```python
from build123d import *

# Parameters (mm, degrees)
EXTRUDE_1_DEPTH     = 130
SKETCH_2_R          = 3
CUT_EXTRUDE_1_DEPTH = 20
SKETCH_9_W          = 50
SKETCH_9_H          = 55
CUT_EXTRUDE_2_DEPTH = 150
SKETCH_10_W         = 100
SKETCH_10_H         = 45
CUT_EXTRUDE_3_DEPTH = 200


with BuildPart() as part:
    # 草图1 → 凸台-拉伸1 (new body)
    with BuildSketch(Plane.XY):
        with BuildLine():
            Line((-450.427662897, 234.022122697), (-950.427662897, 234.022122697))
            Line((-950.427662897, 234.022122697), (-950.427662897, 299.022122697))
            Line((-950.427662897, 299.022122697), (-450.427662897, 299.022122697))
            ThreePointArc((-450.427662897, 299.022122697), (-217.927662897, 66.522122697), (-450.427662897, -165.977877303))
            Line((-450.427662897, -165.977877303), (-700.427662897, -165.977877303))
            Line((-700.427662897, -165.977877303), (-700.427662897, -100.977877303))
            Line((-700.427662897, -100.977877303), (-450.427662897, -100.977877303))
            ThreePointArc((-450.427662897, -100.977877303), (-282.927662897, 66.522122697), (-450.427662897, 234.022122697))
        make_face()
    extrude(amount=EXTRUDE_1_DEPTH)

    # 草图2 → 切除-拉伸1 (cut)
    with BuildSketch(Plane.ZY.offset(950.427662897)):
        with Locations((6, 279.022122697)):
            Circle(SKETCH_2_R)
        with Locations((6, 254.022122697)):
            Circle(SKETCH_2_R)
        with Locations((124, 279.022122697)):
            Circle(SKETCH_2_R)
        with Locations((124, 254.022122697)):
            Circle(SKETCH_2_R)
    extrude(amount=-CUT_EXTRUDE_1_DEPTH, mode=Mode.SUBTRACT)

    # 草图9 → 切除-拉伸2 (cut)
    with BuildSketch(Plane.XY.offset(130)):
        with Locations((-915.427662897, 266.522122697)):
            Rectangle(SKETCH_9_W, SKETCH_9_H)
    extrude(amount=-CUT_EXTRUDE_2_DEPTH, mode=Mode.SUBTRACT)

    # 草图10 → 切除-拉伸3 (cut)
    with BuildSketch(Plane.ZY.offset(950.427662897)):
        with Locations((65, 266.522122697)):
            Rectangle(SKETCH_10_W, SKETCH_10_H)
    extrude(amount=-CUT_EXTRUDE_3_DEPTH, mode=Mode.SUBTRACT)


solid = part.part
```
Geometry: final body of the model. Coordinates: model frame, mm. A direction names the side the tool comes from. Round coordinates to 2 decimals unless told otherwise and drop trailing zeros. Write each loop counter-clockwise with the first axis right and the second up, starting at its lowest first coordinate (ties: lowest second). Pieces come first, ordered by that corner, then holes. Notation, with made-up numbers: (75, -0.75) -> (118, -0.75) arc R26 cw to (118, 15.25) -> close; hole circle Ø3 at (66.5, 50). An arc over 180 degrees is marked (long way). Return JSON: item names as keys, results as strings.
Q1. Section C-C on x = -377.5. Return the cut outline in (y, z), and give its area (3 significant figures).
From the geometry:
{"outline": "(-154.24, 0) -> (-84.27, 0) -> (-84.27, 130) -> (-154.24, 130) -> close; (217.31, 0) -> (287.29, 0) -> (287.29, 130) -> (217.31, 130) -> close", "area": "18,200 mm2"}
Q2. Set-up query: faces 5 (the flat face through (-916, 294.022, 66)), 6 (the flat face through (-821, 244.022, 64)), 7 (the flat face through (-577, -100.978, 64)). Return all of +Z, -Z, +X, -X, +Y, -Y with unobstructed straight access to the full face (end or side cutting, diameter ignored); none if empty.
From the geometry:
{"face 5": "+Z, -Z", "face 6": "-X", "face 7": "+Z, -Z, -X"}
Q3. First-contact query: pin 1 Ø8 at (y, z) = (279.02, 6) entering from +X; pin 2 Ø3.5 at (y, z) = (279.02, 124) entering from +X; pin 3 Ø9.5 at (y, z) = (254.02, 124) entering from +X. Flat tips, straight axial feed; report the tip coordinate or a pass-through.
From the geometry:
{"pin 1": "x = -347.54", "pin 2": "x = -352.24", "pin 3": "x = -306.69"}
Q4. Mould query, pull axis Z, two halves, no side actions, for faces 1 (the flat face through (-821, 266, 115)), 2 (the flat face through (-750.428, 267, 64)), 3 (the flat face through (-528, 240, 0)), 4 (the flat face through (-574, -165.978, 64)). Classes: +Z half, -Z half, draft (parallel to the pull), parting line (faces both ways), or undercut.
From the geometry:
{"face 1": "undercut", "face 2": "undercut", "face 3": "-Z half", "face 4": "draft"}
Q5. Ray query, line 1 (Y direction, x = -942.25, z = 6); line 2 (Y direction, x = -558.5, z = 112); line 3 (Y direction, x = -914.5, z = 10). Return the intervals inside material, ascending.
From the geometry:
{"line 1": "234.02 to 251.02, 257.02 to 276.02, 282.02 to 299.02", "line 2": "-165.98 to -100.98, 234.02 to 299.02", "line 3": "234.02 to 239.02, 294.02 to 299.02"}
Q6. Section A-A on x = -552. Return the cut outline in (y, z), and give its area (3 significant figures).
From the geometry:
{"outline": "(-165.98, 0) -> (-100.98, 0) -> (-100.98, 130) -> (-165.98, 130) -> close; (234.02, 0) -> (299.02, 0) -> (299.02, 130) -> (234.02, 130) -> close", "area": "16,900 mm2"}
Q7. Section D-D on y = 77. Return the cut outline in (x, z).
From the geometry:
{"outline": "(-283.26, 0) -> (-218.16, 0) -> (-218.16, 130) -> (-283.26, 130) -> close"}
Q8. Section B-B on z = 74. Return the cut outline in (x, y), and give its area (3 significant figures).
From the geometry:
{"outline": "(-950.43, 234.02) -> (-450.43, 234.02) arc R167.5 cw to (-450.43, -100.98) -> (-700.43, -100.98) -> (-700.43, -165.98) -> (-450.43, -165.98) arc R232.5 ccw to (-450.43, 299.02) -> (-950.43, 299.02) -> (-950.43, 289.02) -> (-940.43, 289.02) -> (-940.43, 294.02) -> (-890.43, 294.02) -> (-890.43, 289.02) -> (-750.43, 289.02) -> (-750.43, 244.02) -> (-890.43, 244.02) -> (-890.43, 239.02) -> (-940.43, 239.02) -> (-940.43, 244.02) -> (-950.43, 244.02) -> close", "area": "80,100 mm2"}
